from build123d import *

# Parameters (mm, degrees)
BOSS_EXTRUDE1_DEPTH = 45
CUT_EXTRUDE1_DEPTH  = 63.865688575
BOSS_EXTRUDE2_DEPTH = 2.5
BOSS_EXTRUDE3_DEPTH = 2.5
SKETCH5_W           = 0.61
SKETCH5_H           = 4
CUT_EXTRUDE2_DEPTH  = 10


with BuildPart() as part:
    # Sketch1 → Boss-Extrude1 (new body)
    with BuildSketch(Plane(origin=(0, 0, 0), x_dir=(1, 0, 0), z_dir=(0, 1, 0))):
        Polygon((-43.58, 0), (-38.89, 0), (-38.89, 2), (-14.09, 2), (-14.09, 0), (0, 0), (0, 5.28), (-14.09, 5.28), (-14.09, 3.28), (-43.58, 3.28), align=None)
    extrude(amount=BOSS_EXTRUDE1_DEPTH)

    # Sketch2 → Cut-Extrude1 (cut, through all)
    with BuildSketch(Plane.XY):
        Polygon((0, 0), (-43.58, 0), (-43.58, 7.684329819), align=None)
    extrude(amount=-CUT_EXTRUDE1_DEPTH, mode=Mode.SUBTRACT)

    # Sketch3 → Boss-Extrude2 (add)
    with BuildSketch(Plane(origin=(0, 45, 0), x_dir=(1, 0, 0), z_dir=(0, 1, 0))):
        Polygon((-44.97, 4.67), (-44.97, 0.61), (-15.48, 0.61), (-15.48, -1.39), (1.39, -1.39), (1.39, 6.67), (-15.48, 6.67), (-15.48, 4.67), align=None)
    extrude(amount=BOSS_EXTRUDE2_DEPTH)

    # Sketch4 → Boss-Extrude3 (add)
    with BuildSketch(Plane(origin=(0, 47.5, 0), x_dir=(1, 0, 0), z_dir=(0, 1, 0))):
        Polygon((-45.97, 5.67), (-45.97, -0.39), (-16.48, -0.39), (-16.48, -2.39), (2.39, -2.39), (2.39, 7.67), (-16.48, 7.67), (-16.48, 5.67), align=None)
    extrude(amount=BOSS_EXTRUDE3_DEPTH)

    # Sketch5 → Cut-Extrude2 (cut)
    with BuildSketch(Plane.ZY.offset(43.58)):
        with Locations((-0.305, 43)):
            Rectangle(SKETCH5_W, SKETCH5_H)
    extrude(amount=-CUT_EXTRUDE2_DEPTH, mode=Mode.SUBTRACT)


solid = part.part
Input: part model. Units: mm. Frame: model coordinates. A direction names the side the tool comes from. Round coordinates to 2 decimals unless told otherwise and drop trailing zeros. Order: outer loops, then holes, each group sorted by start corner. A loop starts at its lowest first (then second) coordinate and runs counter-clockwise, first axis right, second up.
1. Set-up query: faces 4 (the face through (-29, 23, -3.28)), 5 (the face through (-7, 46, -6.67)), 6 (the face through (0, 22, -3)), 7 (the face through (-14.09, 23, -1)), 8 (the face through (-15.48, 46, 0)). Return all of +Z, -Z, +X, -X, +Y, -Y with unobstructed straight access to the full face (end or side cutting, diameter ignored); none if empty.
The answers:
face 4: -Z, -X, -Y
face 5: -Z, +X, -X, -Y
face 6: +Z, -Z, +X, -Y
face 7: +Z, -Y
face 8: +Z, -X, -Y
2. Material intervals for line 1 (X direction, y = 31.5, z = -0.75); line 2 (Z direction, x = -23, y = 15.5); line 3 (Y direction, x = -35, z = -5.5), sorted ascending.
The answers:
line 1: x = -43.58 to -38.89, -14.09 to 0
line 2: z = -3.28 to -2
line 3: y = 47.5 to 50
3. Mould query, pull axis Y, two halves, no side actions, for faces 1 (the face through (-17, 50, -3)), 2 (the face through (-34, 46, -0.61)), 3 (the face through (-7, 46, 1.39)). Classes: released by +Y, released by -Y, zero draft, split by the parting line, or undercut.
The answers:
face 1: released by +Y
face 2: undercut
face 3: zero draft
4. Cut plane A-A, the plane y = 20. Output: boundary loops of the cut face in (x, z).
The answers:
outline: (-43.58, -3.28) - (-14.09, -3.28) - (-14.09, -5.28) - (0, -5.28) - (0, 0) - (-14.09, 0) - (-14.09, -2) - (-38.89, -2) - (-38.89, 0) - (-43.58, 0) - close
5. Cut plane C-C, the plane x = -25. Output: boundary loops of the cut face in (y, z).
The answers:
outline: (4.41, -3.28) - (45, -3.28) - (45, -4.67) - (47.5, -4.67) - (47.5, -5.67) - (50, -5.67) - (50, 0.39) - (47.5, 0.39) - (47.5, -0.61) - (45, -0.61) - (45, -2) - (4.41, -2) - close
6. Cut plane B-B, the plane x = -32. Output: boundary loops of the cut face in (y, z), then the cut area to 3 significant figures.
The answers:
outline: (5.64, -3.28) - (45, -3.28) - (45, -4.67) - (47.5, -4.67) - (47.5, -5.67) - (50, -5.67) - (50, 0.39) - (47.5, 0.39) - (47.5, -0.61) - (45, -0.61) - (45, -2) - (5.64, -2) - close
area: 75.7 mm2
7. Pin query (flat end, axial travel): P1, Ø1.2, axis at x = -8, y = 46, coming from the -Z side; P2, Ø1.5, axis at x = -10, y = 40.5, coming from the +Z side; P3, Ø1.2, axis at x = -28.5, y = 49.5, coming from the -Z side. Return the tip coordinate at first contact, or that it passes through.
The answers:
P1: stops at z = -6.67
P2: stops at z = 0
P3: stops at z = -5.67
